Geometry check sheet. Reference: the model listing, model coordinates, mm. Give positions to 0.01 mm unless a question says otherwise; leave off trailing zeros. Loops run counter-clockwise (first coordinate to the right, second up) from the corner with the lowest first, then second, coordinate; pieces in that order, holes last. Notation, with made-up numbers: (15.5, 34) -> (68.5, 34) arc R15 ccw to (68.5, 63) -> close; hole circle Ø10 at (-11.5, -23). An arc over 180 degrees is marked (long way). Answer as a JSON object with one key per item and string values.
from build123d import *

# Parameters (mm, degrees)
SKETCH1_W           = 3
SKETCH1_H           = 32
EXTRUDE_THIN1_DEPTH = 300
CUT_EXTRUDE1_DEPTH  = 302.716754589
LPATTERN1_COUNT     = 14
LPATTERN1_PITCH     = 20


with BuildPart() as part:
    # Sketch1 → Extrude-Thin1 (new body)
    with BuildSketch(Plane.XY):
        with Locations((-1.5, -16)):
            Rectangle(SKETCH1_W, SKETCH1_H)
    extrude(amount=EXTRUDE_THIN1_DEPTH)

    # Sketch2 → Cut-Extrude1 (cut, through all)
    with BuildSketch(Plane(origin=(0, 0, 0), x_dir=(0, 0, -1), z_dir=(1, 0, 0))):
        with BuildLine():
            Line((-275, -27), (-275, -32))
            Line((-275, -32), (-285, -32))
            Line((-285, -32), (-285, -27))
            ThreePointArc((-285, -27), (-280, -22), (-275, -27))
        make_face()
    cut_extrude1 = extrude(amount=-CUT_EXTRUDE1_DEPTH, mode=Mode.SUBTRACT)

    # LPattern1: Cut-Extrude1 ×14
    with Locations(*[(0, 0, -i * LPATTERN1_PITCH) for i in range(1, LPATTERN1_COUNT)]):
        add(cut_extrude1, mode=Mode.SUBTRACT)


solid = part.part
1) Draft check along Z on faces 1 (the face through (-3, -16, 148)), 2 (the face through (-1, -22, 280)). Enter one of: pulls with the +Z half, pulls with the -Z half, needs draft (parallel to the pull), parting line crosses it, or undercut.
Geometry check:
{"face 1": "needs draft", "face 2": "undercut"}
2) Section check B-B on z = 140. Record the cut outline in (x, y), plus the area to 3 significant figures.
Geometry check:
{"outline": "(-3, -22) -> (0, -22) -> (0, 0) -> (-3, 0) -> close", "area": "66.0 mm2"}
3) Section check A-A on y = -29.5. Count the separate pieces of the cut face and the enclosed holes in it, plus the area to 3 significant figures.
Geometry check:
{"separate pieces": "15", "enclosed holes": "0", "area": "480 mm2"}
4) Section check C-C on z = 57.5. Record the cut outline in (x, y).
Geometry check:
{"outline": "(-3, -22.67) -> (0, -22.67) -> (0, 0) -> (-3, 0) -> close"}
5) Material ranges on line 1 along Y through (x, z) = (-1.2, 100); line 2 along Y through (x, z) = (-2.4, 124), recorded low to high. Write a range as from..to.
Geometry check:
{"line 1": "y = -22..0", "line 2": "y = -24..0"}
